Geometry check sheet. Reference: the model listing, model coordinates, mm. Face numbers are marked on the shaded views. Coordinates: 2 decimals unless noted, no trailing zeros. Order: outer loops, then holes, each group sorted by start corner. A loop starts at its lowest first (then second) coordinate and runs counter-clockwise, first axis right, second up.
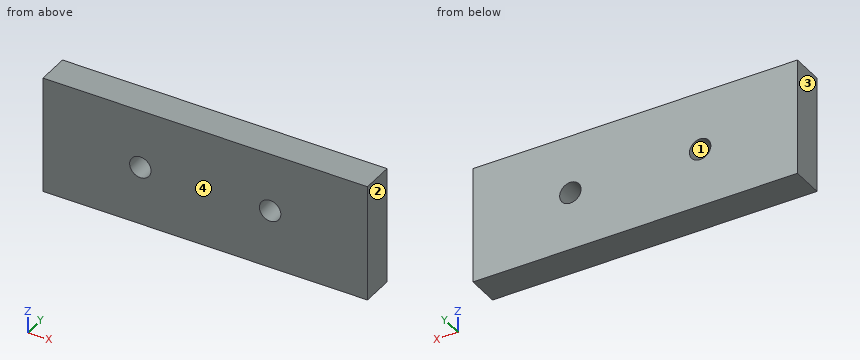
```python
from build123d import *

# Parameters (mm, degrees)
EXTRUDE_1_DEPTH        = 2.5
HOLE_WIZARD_M4_1_D     = 3.3
HOLE_WIZARD_M4_1_DEPTH = 10.1
HOLE_WIZARD_M4_1_TIP   = 0.991420021


with BuildPart() as part:
    # 草图1 → 凸台-拉伸1 (new, symmetric)
    with BuildSketch(Plane(origin=(0, 0, 0), x_dir=(1, 0, 0), z_dir=(0, 1, 0))):
        Polygon((0, 0), (0, -9), (50, -9), (50, 9), (0, 9), align=None)
    extrude(amount=EXTRUDE_1_DEPTH, both=True)

    # M4 螺纹孔1
    with Locations(Plane(origin=(0, 2.5, 0), x_dir=(1, 0, 0), z_dir=(0, 1, 0))):
        with Locations((15, 0), (35, 0)):
            Hole(HOLE_WIZARD_M4_1_D / 2, depth=HOLE_WIZARD_M4_1_DEPTH)
            with Locations((0, 0, -(HOLE_WIZARD_M4_1_DEPTH + HOLE_WIZARD_M4_1_TIP / 2))):  # 118° drill point
                Cone(0, HOLE_WIZARD_M4_1_D / 2, HOLE_WIZARD_M4_1_TIP, mode=Mode.SUBTRACT)


solid = part.part
```
Item 1: Sectioned sample at B-B (x = 35). Record the cut outline in (y, z), and give its area (3 significant figures).
Item 2: Thickness scan on line 1 along Z through (x, y) = (15, 0); line 2 along Z through (x, y) = (33.5, -1.05). Record the ranges inside material, lowest first.
Item 3: Sectioned sample at C-C (y = -1.5). Record the cut outline in (x, z), and give its area (3 significant figures).
Item 4: Sectioned sample at A-A (z = 1). Record the cut outline in (x, y), and give its area (3 significant figures).
Item 5: Sectioned sample at D-D (x = 15.5). Record the cut outline in (y, z), and give its area (3 significant figures).
Item 6: Release check for a two-part mould opening along X. For the marked faces 1, 2, 3 and 4 record: pulls with the +X half, pulls with the -X half, needs draft (parallel to the pull), parting line crosses it, or undercut.
Geometry check:
1. outline: (-2.5, -9) - (2.5, -9) - (2.5, -1.65) - (-2.5, -1.65) - close; (-2.5, 1.65) - (2.5, 1.65) - (2.5, 9) - (-2.5, 9) - close
1. area: 73.5 mm2
2. line 1: z = -9 to -1.65, 1.65 to 9
2. line 2: z = -9 to -0.69, 0.69 to 9
3. outline: (0, -9) - (50, -9) - (50, 9) - (0, 9) - close; hole circle Ø3.3 at (15, 0); hole circle Ø3.3 at (35, 0)
3. area: 883 mm2
4. outline: (0, -2.5) - (13.69, -2.5) - (13.69, 2.5) - (0, 2.5) - close; (16.31, -2.5) - (33.69, -2.5) - (33.69, 2.5) - (16.31, 2.5) - close; (36.31, -2.5) - (50, -2.5) - (50, 2.5) - (36.31, 2.5) - close
4. area: 224 mm2
5. outline: (-2.5, -9) - (2.5, -9) - (2.5, -1.57) - (-2.5, -1.57) - close; (-2.5, 1.57) - (2.5, 1.57) - (2.5, 9) - (-2.5, 9) - close
5. area: 74.3 mm2
6. face 1: undercut
6. face 2: pulls with the +X half
6. face 3: pulls with the -X half
6. face 4: needs draft
